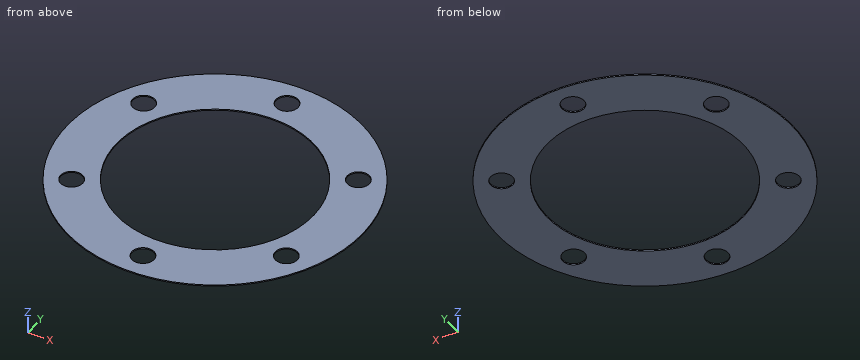
```python
from build123d import *

# Parameters (mm, degrees)
SKETCH1_R           = 60
SKETCH1_R_2         = 40
BOSS_EXTRUDE1_DEPTH = 0.5
SKETCH2_R           = 4.5
CUT_EXTRUDE1_DEPTH  = 85.854286869
CIRPATTERN1_COUNT   = 6


with BuildPart() as part:
    # Sketch1 → Boss-Extrude1 (new body)
    with BuildSketch(Plane.XY):
        Circle(SKETCH1_R)
        Circle(SKETCH1_R_2, mode=Mode.SUBTRACT)
    extrude(amount=BOSS_EXTRUDE1_DEPTH)

    # Sketch2 → Cut-Extrude1 (cut, through all)
    with BuildSketch(Plane.XY.offset(0.5)):
        with Locations((0, 50)):
            Circle(SKETCH2_R)
    cut_extrude1 = extrude(amount=-CUT_EXTRUDE1_DEPTH, mode=Mode.SUBTRACT)

    # CirPattern1: Cut-Extrude1 ×6 about axis
    cirpattern1_axis = Axis((0, 0, 0), (0, 0, 1))
    for i in range(1, CIRPATTERN1_COUNT):
        add(cut_extrude1.rotate(cirpattern1_axis, i * 360 / CIRPATTERN1_COUNT), mode=Mode.SUBTRACT)


solid = part.part
```
Source: CAD feature listing. Evaluate the final solid. Frame: model axes, mm. Coordinates: 2 decimals unless noted, no trailing zeros. Loops run counter-clockwise (first coordinate to the right, second up) from the corner with the lowest first, then second, coordinate; pieces in that order, holes last. Notation, with made-up numbers: (39, -1) - (50, -1) arc R24 cw to (50, 27) - close; hole circle Ø2 at (15, 68). An arc over 180 degrees is marked (long way). Answer as CSV lines item,"result".
1. Section D-D (z = 0.4). Return loops of the section in (x, y), then the cut area to 3 significant figures.
Established:
outline,"circle Ø120 at (0, 0); hole circle Ø9 at (-43.3, -25); hole circle Ø9 at (-43.3, 25); hole circle Ø80 at (0, 0); hole circle Ø9 at (0, -50); hole circle Ø9 at (0, 50); hole circle Ø9 at (43.3, -25); hole circle Ø9 at (43.3, 25)"
area,"5,900 mm2"
2. Section C-C (y = -26). Return loops of the section in (x, z), then the cut area to 3 significant figures.
Established:
outline,"(-54.07, 0) - (-47.69, 0) - (-47.69, 0.5) - (-54.07, 0.5) - close; (-38.91, 0) - (-30.4, 0) - (-30.4, 0.5) - (-38.91, 0.5) - close; (30.4, 0) - (38.91, 0) - (38.91, 0.5) - (30.4, 0.5) - close; (47.69, 0) - (54.07, 0) - (54.07, 0.5) - (47.69, 0.5) - close"
area,"14.9 mm2"
3. Ray query, line 1 (Y direction, x = 0, z = 0.45); line 2 (X direction, y = -26.5, z = 0.35); line 3 (Y direction, x = -47, z = 0.2). Return the intervals inside material, ascending.
Established:
line 1,"y = -60 to -54.5, -45.5 to -40, 40 to 45.5, 54.5 to 60"
line 2,"x = -53.83 to -47.54, -39.06 to -29.96, 29.96 to 39.06, 47.54 to 53.83"
line 3,"y = -37.3 to -27.56, -22.44 to 22.44, 27.56 to 37.3"
4. Section A-A (y = 6.5). Return loops of the section in (x, z), then the cut area to 3 significant figures.
Established:
outline,"(-59.65, 0) - (-39.47, 0) - (-39.47, 0.5) - (-59.65, 0.5) - close; (39.47, 0) - (59.65, 0) - (59.65, 0.5) - (39.47, 0.5) - close"
area,"20.2 mm2"
5. Contact query for flat-ended pins moving along their axis: pin 1 (11.5 mm diameter, centred on x = 0, y = 50, fed in from -Z); pin 2 (7 mm diameter, centred on x = -43.3, y = 25, fed in from +Z). Output: stop coordinate, or through.
Established:
pin 1,"stops at z = 0"
pin 2,"passes through"
6. Section B-B (x = 20). Return loops of the section in (y, z), then the cut area to 3 significant figures.
Established:
outline,"(-56.57, 0) - (-34.64, 0) - (-34.64, 0.5) - (-56.57, 0.5) - close; (34.64, 0) - (56.57, 0) - (56.57, 0.5) - (34.64, 0.5) - close"
area,"21.9 mm2"
